Can you work these out from the model? Positions are in its coordinate system, mm. A direction names the side the tool comes from. Round coordinates to 2 decimals unless told otherwise and drop trailing zeros. Write each loop counter-clockwise with the first axis right and the second up, starting at its lowest first coordinate (ties: lowest second). Pieces come first, ordered by that corner, then holes. Notation, with made-up numbers: M 25,63 L 36,63 A31 ccw 36,98 Z; hole C 36.5,58 d10. An arc over 180 degrees is marked long. Answer in a Markdown table with one row per item. Add a question column.
(1) For faces 1 (the face through (-11.99, 0.53, -453.5)), 2 (the face through (-11.99, 0.53, -18)), 3 (the face through (0, 0, 0)), which set-ups out of +Z, -Z, +X, -X, +Y, -Y let a thin tool reach every point of the face, with its end or its side?
(2) Suppose I cut it at C-C, the plane z = -518. Write out the boundary of the cut face in (x, y), then the cut area to 3 significant figures.
(3) If I drill on probe 1 along Y at (x, z) = (9.75, -407.5); probe 2 along Z at (x, y) = (3.25, -9.5); probe 3 along Z at (x, y) = (11.25, 4), over which ranges is the centre line in solid material (lowest first)?
(4) Suppose I cut it at B-B, the plane z = -219. Write out the boundary of the cut face in (x, y), then the cut area to 3 significant figures.
(5) I'm going to push flat-ended pins straight in: pin 1 (3 mm diameter, centred on y = 1.5, z = -508, fed in from -X); pin 2 (1.5 mm diameter, centred on y = 8.5, z = -558, fed in from -X); pin 3 (6 mm diameter, centred on x = 9, z = -101.5, fed in from +Y). Where does each tip first touch, or does it pass through?
from build123d import *

# Parameters (mm, degrees)
SKETCH1_R           = 12
BOSS_EXTRUDE1_DEPTH = 472
SKETCH2_R           = 11
BOSS_EXTRUDE2_DEPTH = 100
SKETCH4_R           = 14
BOSS_EXTRUDE3_DEPTH = 400
CHAMFER1_SIZE       = 1
CHAMFER2_SIZE       = 0.5
CHAMFER3_SIZE       = 0.5
SKETCH5_R           = 20
SKETCH5_R_2         = 10
CUT_EXTRUDE1_DEPTH  = 36
CUT_EXTRUDE2_DEPTH  = 573.538426658
CHAMFER4_SIZE       = 0.5


with BuildPart() as part:
    # Sketch1 → Boss-Extrude1 (new body)
    with BuildSketch(Plane.XY):
        Circle(SKETCH1_R)
    extrude(amount=-BOSS_EXTRUDE1_DEPTH)

    # Sketch2 → Boss-Extrude2 (add)
    with BuildSketch(Plane(origin=(0, 0, -472), x_dir=(-1, 0, 0), z_dir=(0, 0, -1))):
        Circle(SKETCH2_R)
    extrude(amount=BOSS_EXTRUDE2_DEPTH)

    # Sketch4 → Boss-Extrude3 (add)
    with BuildSketch(Plane.XY.offset(-36)):
        Circle(SKETCH4_R)
    extrude(amount=-BOSS_EXTRUDE3_DEPTH)

    # Chamfer1
    chamfer1_edges = [part.edges().sort_by_distance(p)[0] for p in [
        (-14, 0, -36),
        (-14, 0, -436),
    ]]
    chamfer(chamfer1_edges, length=CHAMFER1_SIZE)

    # Chamfer2
    chamfer2_edges = [part.edges().sort_by_distance(p)[0] for p in [
        (-12, 0, 0),
    ]]
    chamfer(chamfer2_edges, length=CHAMFER2_SIZE)

    # Chamfer3
    chamfer3_edges = [part.edges().sort_by_distance(p)[0] for p in [
        (-12, 0, -472),
    ]]
    chamfer(chamfer3_edges, length=CHAMFER3_SIZE)

    # Sketch5 → Cut-Extrude1 (cut)
    with BuildSketch(Plane(origin=(0, 0, -572), x_dir=(-1, 0, 0), z_dir=(0, 0, -1))):
        Circle(SKETCH5_R)
        Circle(SKETCH5_R_2, mode=Mode.SUBTRACT)
    extrude(amount=-CUT_EXTRUDE1_DEPTH, mode=Mode.SUBTRACT)

    # Sketch6 → Cut-Extrude2 (cut, through all)
    with BuildSketch(Plane(origin=(0, 6.5, 0), x_dir=(1, 0, 0), z_dir=(0, 1, 0))):
        with BuildLine():
            Line((3, 576.648489628), (3, 541))
            ThreePointArc((3, 541), (0, 538), (-3, 541))
            Line((-3, 541), (-3, 576.648489628))
            ThreePointArc((-3, 576.648489628), (0, 579.648489628), (3, 576.648489628))
        make_face()
    extrude(amount=CUT_EXTRUDE2_DEPTH, mode=Mode.SUBTRACT)

    # Chamfer4
    chamfer4_edges = [part.edges().sort_by_distance(p)[0] for p in [
        (5.916079783, -8.062257748, -572),
    ]]
    chamfer(chamfer4_edges, length=CHAMFER4_SIZE)


solid = part.part
Calculated:
| question | item | result |
|---|---|---|
| 1 | face 1 | -Z |
| 1 | face 2 | +Z |
| 1 | face 3 | +Z, +X, -X, +Y, -Y |
| 2 | outline | C 0,0 d22 |
| 2 | area | 380 mm² |
| 3 | probe 1 | -10.05 to 10.05 |
| 3 | probe 2 | -536 to 0 |
| 3 | probe 3 | -471.56 to -0.44 |
| 4 | outline | C 0,0 d28 |
| 4 | area | 616 mm² |
| 5 | pin 1 | x = -11 |
| 5 | pin 2 | x = -6.32 |
| 5 | pin 3 | y = 12.65 |
